The listing builds one solid part. Answer for the finished solid, in the listing's coordinates (mm). Coordinates: 2 decimals unless noted, no trailing zeros. Loops run counter-clockwise (first coordinate to the right, second up) from the corner with the lowest first, then second, coordinate; pieces in that order, holes last. Notation, with made-up numbers: (15, 25.25) - (55, 25.25) arc R18 cw to (55, 35.25) - close; hole circle Ø11 at (63, -15.5). An arc over 180 degrees is marked (long way). Write each question's results on one line, items separated by ' | '. Start each with the question number.
(1) Find section C-C on z = 0.1. Determine the outline of the cut face in (x, y), then the cut area to 3 significant figures.
(2) Find section D-D on z = -2. Determine the outline of the cut face in (x, y).
(3) Given pin 1 Ø2 at (x, z) = (0.5, 0.5) entering from -Y; pin 2 Ø2 at (y, z) = (3, 1.5) entering from +X, each flat-ended and moving along its own axis, determine where each tip first touches the part or whether it passes through.
(4) Determine the mould class of faces 1 (the cylindrical face through (0.466, 3.451, 1.478)), 2 (the flat face through (2.414, 3.451, 1.42)), 3 (the flat face through (1.4, 0, 1.2)) for opening direction X: released by +X, released by -X, zero draft, split by the parting line, or undercut.
(5) Find section A-A on x = 0. Determine the outline of the cut face in (y, z).
(6) Find section B-B on y = 6.5. Determine the outline of the cut face in (x, z), then the cut area to 3 significant figures.
(7) Consider line 1 (Z direction, x = -0.5, y = 1.75); line 2 (X direction, y = 3.5, z = -0.7); line 3 (X direction, y = 5.75, z = 0.25). Determine where each line is inside the solid, lowest interval first. Write a range as from..to.
from build123d import *

# Parameters (mm, degrees)
SKETCH_1_R      = 1.55
EXTRUDE_1_DEPTH = 7


with BuildPart() as part:
    # 草图1 → 凸台-拉伸1 (new body)
    with BuildSketch(Plane(origin=(0, 0, 0), x_dir=(1, 0, 0), z_dir=(0, 1, 0))):
        Polygon((1.616580754, -2.8), (3.233161507, 0), (1.616580754, 2.8), (-1.616580754, 2.8), (-3.233161507, 0), (-1.616580754, -2.8), align=None)
        with Locations(Location((0, 0, 0), (0, 0, 270))):
            Circle(SKETCH_1_R, mode=Mode.SUBTRACT)
    extrude(amount=EXTRUDE_1_DEPTH)


solid = part.part
Values:
1) outline: (-3.18, 0) - (-1.55, 0) - (-1.55, 7) - (-3.18, 7) - close; (1.55, 0) - (3.18, 0) - (3.18, 7) - (1.55, 7) - close | area: 22.8 mm²
2) outline: (-2.08, 0) - (2.08, 0) - (2.08, 7) - (-2.08, 7) - close
3) pin 1: stops at y = 0 | pin 2: stops at x = 2.94
4) face 1: undercut | face 2: released by +X | face 3: zero draft
5) outline: (0, -2.8) - (7, -2.8) - (7, -1.55) - (0, -1.55) - close; (0, 1.55) - (7, 1.55) - (7, 2.8) - (0, 2.8) - close
6) outline: (-3.23, 0) - (-1.62, -2.8) - (1.62, -2.8) - (3.23, 0) - (1.62, 2.8) - (-1.62, 2.8) - close; hole circle Ø3.1 at (0, 0) | area: 19.6 mm²
7) line 1: z = -2.8..-1.47, 1.47..2.8 | line 2: x = -2.83..-1.38, 1.38..2.83 | line 3: x = -3.09..-1.53, 1.53..3.09
